For this review, take the finished solid that the model builds, in its own axes (mm). Face numbers are marked on the shaded views. A direction names the side the tool comes from. Coordinates: 2 decimals unless noted, no trailing zeros. Order: outer loops, then holes, each group sorted by start corner. A loop starts at its lowest first (then second) coordinate and runs counter-clockwise, first axis right, second up. Notation, with made-up numbers: (-7.5, -33) -> (51.5, -33) arc R34 cw to (51.5, 2) -> close; hole circle Ø11 at (39.5, 37.25). An arc over 180 degrees is marked (long way). Answer as a JSON object with one key per item and string values. Group by question number.
1) For pin 1 (13.5 mm diameter, centred on x = -45, z = -0.5, fed in from +Y); pin 2 (5 mm diameter, centred on y = 70.5, z = 0, fed in from +X); pin 3 (11 mm diameter, centred on y = 141, z = 35, fed in from -X), all flat-tipped, find the tip position at first contact; note any pin that passes through.
2) Add section C-C, the plane y = 139.5. Write out the cut boundary in (x, z).
3) Wall thickness on L1, parallel to X at y = 34, z = 0; L2, parallel to Y at x = -21.5, z = -7; L3, parallel to Z at x = 32, y = 27: over which ranges is each line inside the solid? List them lowest first.
4) Add section A-A, the plane x = 10.5. Write out the cut boundary in (y, z).
5) Machinability: for the marked faces 1, 2 and 3, which of the approach directions +Z, -Z, +X, -X, +Y, -Y give a long, thin tool a straight path to every point of the face, cutting with its end or side? Answer none if there is none.
6) Add section B-B, the plane z = -21. Write out the cut boundary in (x, y), then the cut area to 3 significant figures.
7) Add section D-D, the plane x = 37. Write out the cut boundary in (y, z).
8) Draft analysis for pull direction X (two halves, no side actions). For the marked faces 4, 5 and 6, state which applies: +X half, -X half, draft (parallel to the pull), parting line (faces both ways), or undercut.
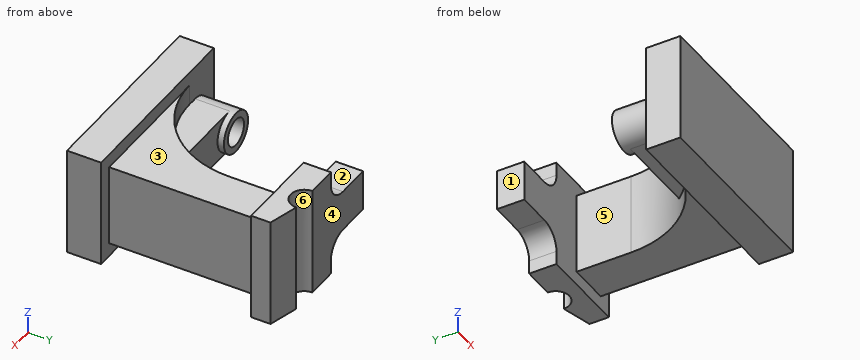
from build123d import *

# Parameters (mm, degrees)
BRACKET_BODY_DEPTH          = 40
BASE_RECESS_SKETCH_W        = 10
BASE_RECESS_SKETCH_H        = 110
BASE_RECESS_CUT_DEPTH       = 207.215906273
CRADLE_GROOVE_R15_DEPTH     = 80
TOP_CHAMFER_CUT_15DEG_DEPTH = 80
PIN_BOSS_SKETCH_R           = 15
PIN_BOSS_SKETCH_R_2         = 10
PIN_BOSS_DEPTH              = 55
CURVED_WEB_DEPTH            = 15
PIN_START                   = -25
PIN_BORE_SKETCH_R           = 10
PIN_BORE_20_DEPTH           = 25


with BuildPart() as part:
    # Bracket Profile Sketch → Bracket Body (new, symmetric)
    with BuildSketch(Plane.XY):
        with BuildLine():
            Line((-40, 25), (60, 25))
            Line((60, 25), (60, 135))
            Line((60, 135), (70, 135))
            Line((70, 135), (70, 155))
            Line((70, 155), (48, 155))
            ThreePointArc((48, 155), (38, 145), (28, 155))
            Line((28, 155), (-35, 155))
            Line((-35, 155), (-35, 135))
            Line((-35, 135), (30, 135))
            Line((30, 135), (30, 95))
            ThreePointArc((30, 95), (9.497474683, 45.502525317), (-40, 25))
        make_face()
        Polygon((-70, 25), (-70, 0), (0, 0), (70, 0), (70, 25), align=None)
    extrude(amount=BRACKET_BODY_DEPTH, both=True)

    # Base Recess Sketch → Base Recess Cut (cut, through all)
    with BuildSketch(Plane(origin=(60, 0, 0), x_dir=(0, 0, -1), z_dir=(1, 0, 0))):
        with Locations((35, 80)):
            Rectangle(BASE_RECESS_SKETCH_W, BASE_RECESS_SKETCH_H)
        with Locations((-35, 80)):
            Rectangle(BASE_RECESS_SKETCH_W, BASE_RECESS_SKETCH_H)
    extrude(amount=-BASE_RECESS_CUT_DEPTH, mode=Mode.SUBTRACT)

    # Cradle Groove Sketch → Cradle Groove R15 (cut)
    with BuildSketch(Plane(origin=(0, 155, 0), x_dir=(1, 0, 0), z_dir=(0, 1, 0))):
        with BuildLine():
            Line((-35, 40), (-35, 15))
            Line((-35, 15), (-10, 15))
            ThreePointArc((-10, 15), (0.606601718, 19.393398282), (5, 30))
            Line((5, 30), (5, 40))
            Line((5, 40), (-35, 40))
        make_face()
        with BuildLine():
            Line((-10, -15), (-35, -15))
            Line((-35, -15), (-35, -40))
            Line((-35, -40), (5, -40))
            Line((5, -40), (5, -30))
            ThreePointArc((5, -30), (0.606601718, -19.393398282), (-10, -15))
        make_face()
    extrude(amount=-CRADLE_GROOVE_R15_DEPTH, mode=Mode.SUBTRACT)

    # Top Chamfer Sketch → Top Chamfer Cut 15deg (cut)
    with BuildSketch(Plane.XY.offset(40)):
        Polygon((48, 155), (70, 149.105117767), (70, 155), align=None)
    extrude(amount=-TOP_CHAMFER_CUT_15DEG_DEPTH, mode=Mode.SUBTRACT)

    # Pin Boss Sketch → Pin Boss (add)
    with BuildSketch(Plane(origin=(0, 0, 0), x_dir=(1, 0, 0), z_dir=(0, 1, 0))):
        with Locations(Location((-46.735177318, 0, 0), (0, 0, 63.319698917))):
            Circle(PIN_BOSS_SKETCH_R)
        with Locations(Location((-46.735177318, 0, 0), (0, 0, 47.660850918))):
            Circle(PIN_BOSS_SKETCH_R_2, mode=Mode.SUBTRACT)
    extrude(amount=PIN_BOSS_DEPTH)

    # Curved Web Sketch → Curved Web (add, symmetric)
    with BuildSketch(Plane.XY):
        with BuildLine():
            Line((-46.735177318, 25.324772074), (-46.735177318, 50.324772074))
            Line((-46.735177318, 50.324772074), (13.889924938, 50.324772074))
            ThreePointArc((13.889924938, 50.324772074), (-13.314000754, 30.286342676), (-46.735177318, 25.324772074))
        make_face()
    extrude(amount=CURVED_WEB_DEPTH, both=True)

    # Pin Bore Sketch → Pin Bore Ø20 (cut)
    with BuildSketch(Plane(origin=(0, 50.324772074, 0), x_dir=(1, 0, 0), z_dir=(0, 1, 0)).offset(PIN_START)):
        with Locations(Location((-46.735177318, 0, 0), (0, 0, 270))):
            Circle(PIN_BORE_SKETCH_R)
    extrude(amount=PIN_BORE_20_DEPTH, mode=Mode.SUBTRACT)


solid = part.part
Output values:
{
 "1": {"pin 1": "stops at y = 25.32", "pin 2": "stops at x = 60", "pin 3": "stops at x = 4.99"},
 "2": {"outline": "(-35, -15) -> (-10, -15) arc R15 cw to (5, -30) -> (5, -40) -> (70, -40) -> (70, 40) -> (5, 40) -> (5, 30) arc R15 cw to (-10, 15) -> (-35, 15) -> close"},
 "3": {"L1": "x = -61.74 to -56.74, -36.74 to 60", "L2": "y = 0 to 50.32, 135 to 155", "L3": "z = -30 to 30"},
 "4": {"outline": "(0, -40) -> (25, -40) -> (25, -30) -> (46.53, -30) -> (46.53, -15) -> (50.32, -15) -> (50.32, 15) -> (46.53, 15) -> (46.53, 30) -> (25, 30) -> (25, 40) -> (0, 40) -> close; (135, -40) -> (155, -40) -> (155, 40) -> (135, 40) -> close"},
 "5": {"face 1": "+Z, -Z, -X, +Y", "face 2": "+Z, -X, +Y", "face 3": "+Z, +X, -X"},
 "6": {"outline": "(-70, 0) -> (70, 0) -> (70, 25) -> (60, 25) -> (60, 135) -> (70, 135) -> (70, 149.11) -> (48, 155) arc R10 cw to (28, 155) -> (2, 155) -> (2, 135) -> (30, 135) -> (30, 95) arc R70 cw to (-40, 25) -> (-70, 25) -> close", "area": "8,990 mm²"},
 "7": {"outline": "(0, -40) -> (25, -40) -> (25, -30) -> (135, -30) -> (135, -40) -> (145.05, -40) -> (145.05, 40) -> (135, 40) -> (135, 30) -> (25, 30) -> (25, 40) -> (0, 40) -> close"},
 "8": {"face 4": "draft", "face 5": "-X half", "face 6": "undercut"}
}
